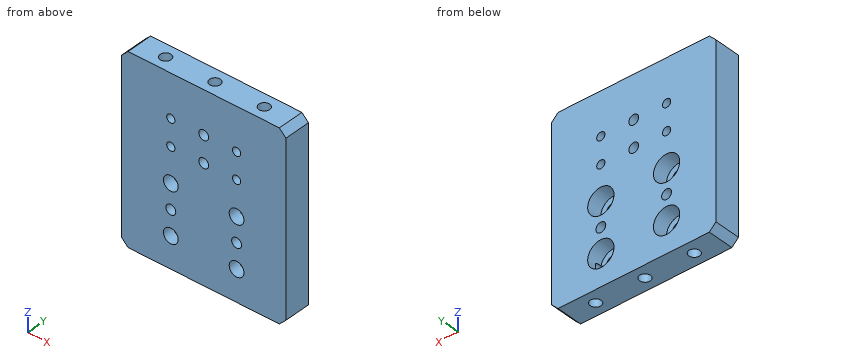
from build123d import *

# Parameters (mm, degrees)
SKETCH_1_W                = 50
SKETCH_1_H                = 56
EXTRUDE_1_DEPTH           = 8
HOLE_WIZARD_M4_1_D        = 3.3
HOLE_WIZARD_M4_1_DEPTH    = 10.1
HOLE_WIZARD_M4_1_TIP      = 0.991420021
CHAMFER_1_SIZE            = 2
HOLE_WIZARD_M4_2_D        = 3.3
HOLE_WIZARD_M4_2_DEPTH    = 10.1
HOLE_WIZARD_M4_2_TIP      = 0.991420021
MM_1_D                    = 3
MM_1_DEPTH                = 12.4
MM_1_TIP                  = 0.901290929
HOLE_WIZARD_M3_1_D        = 2.5
HOLE_WIZARD_M3_1_DEPTH    = 15
HOLE_WIZARD_M3_1_TIP      = 0.751075774
MM_2_D                    = 3
MM_2_DEPTH                = 15
MM_2_TIP                  = 0.901290929
HOLE_WIZARD_1_D           = 4.5
HOLE_WIZARD_1_DEPTH       = 15
HOLE_WIZARD_1_CBORE_D     = 8
HOLE_WIZARD_1_CBORE_DEPTH = 4.6
HOLE_WIZARD_1_TIP         = 1.351936393
HOLE_WIZARD_2_D           = 4.5
HOLE_WIZARD_2_DEPTH       = 15
HOLE_WIZARD_2_CBORE_D     = 8
HOLE_WIZARD_2_CBORE_DEPTH = 4.6
HOLE_WIZARD_2_TIP         = 1.351936393
MM_3_D                    = 3
MM_3_DEPTH                = 15
MM_3_TIP                  = 0.901290929
CHAMFER_2_SIZE            = 2


with BuildPart() as part:
    # 草图1 → 凸台-拉伸1 (new body)
    with BuildSketch(Plane(origin=(0, 0, 0), x_dir=(1, 0, 0), z_dir=(0, 1, 0))):
        Rectangle(SKETCH_1_W, SKETCH_1_H)
    extrude(amount=EXTRUDE_1_DEPTH)

    # M4 螺纹孔1
    with Locations(Plane.XY.offset(28)):
        with Locations((15, 4), (0, 4), (-15, 4)):
            Hole(HOLE_WIZARD_M4_1_D / 2, depth=HOLE_WIZARD_M4_1_DEPTH)
            with Locations((0, 0, -(HOLE_WIZARD_M4_1_DEPTH + HOLE_WIZARD_M4_1_TIP / 2))):  # 118° drill point
                Cone(0, HOLE_WIZARD_M4_1_D / 2, HOLE_WIZARD_M4_1_TIP, mode=Mode.SUBTRACT)

    # 倒角1
    chamfer_1_edges = [part.edges().sort_by_distance(p)[0] for p in [
        (25, 4, 28),
        (-25, 4, 28),
    ]]
    chamfer(chamfer_1_edges, length=CHAMFER_1_SIZE)

    # M4 螺纹孔2
    with Locations(Plane(origin=(0, 0, -28), x_dir=(-1, 0, 0), z_dir=(0, 0, -1))):
        with Locations((-15, 4), (0, 4), (15, 4)):
            Hole(HOLE_WIZARD_M4_2_D / 2, depth=HOLE_WIZARD_M4_2_DEPTH)
            with Locations((0, 0, -(HOLE_WIZARD_M4_2_DEPTH + HOLE_WIZARD_M4_2_TIP / 2))):  # 118° drill point
                Cone(0, HOLE_WIZARD_M4_2_D / 2, HOLE_WIZARD_M4_2_TIP, mode=Mode.SUBTRACT)

    # 大小mm 暗销孔1
    with Locations(Plane(origin=(0, 0, 0), x_dir=(-1, 0, 0), z_dir=(0, -1, 0))):
        with Locations((0, -7), (0, -15)):
            Hole(MM_1_D / 2, depth=MM_1_DEPTH)
            with Locations((0, 0, -(MM_1_DEPTH + MM_1_TIP / 2))):  # 118° drill point
                Cone(0, MM_1_D / 2, MM_1_TIP, mode=Mode.SUBTRACT)

    # M3 螺纹孔1
    with Locations(Plane(origin=(0, 0, 0), x_dir=(-1, 0, 0), z_dir=(0, -1, 0))):
        with Locations((-10, -7), (10, -7), (-10, -15), (10, -15)):
            Hole(HOLE_WIZARD_M3_1_D / 2, depth=HOLE_WIZARD_M3_1_DEPTH)
            with Locations((0, 0, -(HOLE_WIZARD_M3_1_DEPTH + HOLE_WIZARD_M3_1_TIP / 2))):  # 118° drill point
                Cone(0, HOLE_WIZARD_M3_1_D / 2, HOLE_WIZARD_M3_1_TIP, mode=Mode.SUBTRACT)

    # 大小mm 暗销孔2
    with Locations(Plane(origin=(0, 8, 0), x_dir=(1, 0, 0), z_dir=(0, 1, 0))):
        with Locations((-10, 11)):
            Hole(MM_2_D / 2, depth=MM_2_DEPTH)
            with Locations((0, 0, -(MM_2_DEPTH + MM_2_TIP / 2))):  # 118° drill point
                Cone(0, MM_2_D / 2, MM_2_TIP, mode=Mode.SUBTRACT)

    # 打孔尺寸(%根据)内六角圆柱头螺钉的类型1
    with Locations(Plane(origin=(0, 8, 0), x_dir=(1, 0, 0), z_dir=(0, 1, 0))):
        with Locations((-10, 18.5), (-10, 3.5)):
            CounterBoreHole(HOLE_WIZARD_1_D / 2, HOLE_WIZARD_1_CBORE_D / 2, HOLE_WIZARD_1_CBORE_DEPTH, depth=HOLE_WIZARD_1_DEPTH)
            with Locations((0, 0, -(HOLE_WIZARD_1_DEPTH + HOLE_WIZARD_1_TIP / 2))):  # 118° drill point
                Cone(0, HOLE_WIZARD_1_D / 2, HOLE_WIZARD_1_TIP, mode=Mode.SUBTRACT)

    # 打孔尺寸(%根据)内六角圆柱头螺钉的类型2
    with Locations(Plane(origin=(0, 8, 0), x_dir=(1, 0, 0), z_dir=(0, 1, 0))):
        with Locations((10, 18.5), (10, 3.5)):
            CounterBoreHole(HOLE_WIZARD_2_D / 2, HOLE_WIZARD_2_CBORE_D / 2, HOLE_WIZARD_2_CBORE_DEPTH, depth=HOLE_WIZARD_2_DEPTH)
            with Locations((0, 0, -(HOLE_WIZARD_2_DEPTH + HOLE_WIZARD_2_TIP / 2))):  # 118° drill point
                Cone(0, HOLE_WIZARD_2_D / 2, HOLE_WIZARD_2_TIP, mode=Mode.SUBTRACT)

    # 大小mm 暗销孔3
    with Locations(Plane(origin=(0, 8, 0), x_dir=(1, 0, 0), z_dir=(0, 1, 0))):
        with Locations((10, 11)):
            Hole(MM_3_D / 2, depth=MM_3_DEPTH)
            with Locations((0, 0, -(MM_3_DEPTH + MM_3_TIP / 2))):  # 118° drill point
                Cone(0, MM_3_D / 2, MM_3_TIP, mode=Mode.SUBTRACT)

    # 倒角2
    chamfer_2_edges = [part.edges().sort_by_distance(p)[0] for p in [
        (-25, 4, -28),
        (25, 4, -28),
    ]]
    chamfer(chamfer_2_edges, length=CHAMFER_2_SIZE)


solid = part.part
Input: part model. Units: mm. Frame: model coordinates. Give positions to 0.01 mm unless a question says otherwise; leave off trailing zeros. Order: outer loops, then holes, each group sorted by start corner. A loop starts at its lowest first (then second) coordinate and runs counter-clockwise, first axis right, second up. Notation, with made-up numbers: (-30.75, -15) -> (0.25, -15) arc R28 ccw to (0.25, 20) -> close; hole circle Ø2 at (13, 84.25). An arc over 180 degrees is marked (long way). Use one line per item in the form item = value.
1) Section B-B, the plane x = -10. Count the separate pieces of the cut face and the enclosed holes in it, and give its area (3 significant figures).
Response values:
separate_pieces = 6
enclosed_holes = 0
area = 280 mm^2
2) Section A-A, the plane z = -3.5. Return loops of the section in (x, y).
Response values:
outline = (-25, 0) -> (-12.25, 0) -> (-12.25, 3.4) -> (-14, 3.4) -> (-14, 8) -> (-25, 8) -> close; (-7.75, 0) -> (7.75, 0) -> (7.75, 3.4) -> (6, 3.4) -> (6, 8) -> (-6, 8) -> (-6, 3.4) -> (-7.75, 3.4) -> close; (12.25, 0) -> (25, 0) -> (25, 8) -> (14, 8) -> (14, 3.4) -> (12.25, 3.4) -> close
3) First-contact query: pin 1 Ø2.5 at (x, z) = (-10, -11) entering from +Y; pin 2 Ø3 at (x, z) = (10, 7) entering from +Y; pin 3 Ø2.5 at (x, z) = (-11, -1.5) entering from +Y; pin 4 Ø3 at (x, y) = (-15, 4) entering from +Z. Flat tips, straight axial feed; report the tip coordinate or a pass-through.
Response values:
pin_1 = through
pin_2 = 8
pin_3 = 3.4
pin_4 = 17.81
4) Section D-D, the plane z = -11. Return loops of the section in (x, y), and give its area (3 significant figures).
Response values:
outline = (-25, 0) -> (-11.5, 0) -> (-11.5, 8) -> (-25, 8) -> close; (-8.5, 0) -> (8.5, 0) -> (8.5, 8) -> (-8.5, 8) -> close; (11.5, 0) -> (25, 0) -> (25, 8) -> (11.5, 8) -> close
area = 352 mm^2
5) Line query: probe 1 along Z at (x, y) = (-10, 4.5); probe 2 along X at (y, z) = (1.5, -18.5); probe 3 along X at (y, z) = (4, 23.5). Output: solid intervals per line, ascending.
Response values:
probe_1 = -28 to -22.5, -14.5 to -12.5, -9.5 to -7.5, 0.5 to 5.75, 8.25 to 13.75, 16.25 to 28
probe_2 = -25 to -12.25, -7.75 to 7.75, 12.25 to 25
probe_3 = -25 to -16.65, -13.35 to -1.65, 1.65 to 13.35, 16.65 to 25
